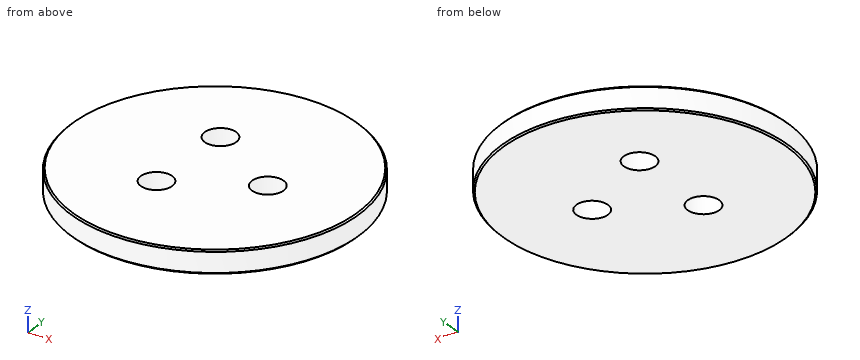
from build123d import *

# Parameters (mm, degrees)
SKETCH1_R           = 100
BOSS_EXTRUDE1_DEPTH = 16
SKETCH2_R           = 11
CUT_EXTRUDE1_DEPTH  = 143.323574997
CIRPATTERN1_COUNT   = 3
CHAMFER1_SIZE       = 1


with BuildPart() as part:
    # Sketch1 → Boss-Extrude1 (new body)
    with BuildSketch(Plane.XY):
        Circle(SKETCH1_R)
    extrude(amount=BOSS_EXTRUDE1_DEPTH)

    # Sketch2 → Cut-Extrude1 (cut, through all)
    with BuildSketch(Plane.XY.offset(16)):
        with Locations((37.5, 0)):
            Circle(SKETCH2_R)
    cut_extrude1 = extrude(amount=-CUT_EXTRUDE1_DEPTH, mode=Mode.SUBTRACT)

    # CirPattern1: Cut-Extrude1 ×3 about axis
    cirpattern1_axis = Axis((0, 0, 0), (0, 0, 1))
    for i in range(1, CIRPATTERN1_COUNT):
        add(cut_extrude1.rotate(cirpattern1_axis, i * 360 / CIRPATTERN1_COUNT), mode=Mode.SUBTRACT)

    # Chamfer1
    chamfer1_edges = [part.edges().sort_by_distance(p)[0] for p in [
        (-100, 0, 0),
        (-100, 0, 16),
    ]]
    chamfer(chamfer1_edges, length=CHAMFER1_SIZE)


solid = part.part
Part model, mm, in its own coordinate system. Give positions to 0.01 mm unless a question says otherwise; leave off trailing zeros. Order: outer loops, then holes, each group sorted by start corner. A loop starts at its lowest first (then second) coordinate and runs counter-clockwise, first axis right, second up. Notation, with made-up numbers: (31.5, -8.5) - (80.5, -8.5) arc R18 ccw to (80.5, 1.5) - close; hole circle Ø3 at (-35.75, 56). An arc over 180 degrees is marked (long way). Use a Markdown table: item, result.
1) Flat gauge pins, fed straight in: P1, Ø3, axis at y = -22.5, z = 2, coming from the +X side; P2, Ø1.5, axis at y = -14.5, z = 6.5, coming from the +X side; P3, Ø1.5, axis at x = 25.5, z = 9, coming from the -Y side; P4, Ø20, axis at x = -18.75, y = -32.48, coming from the +Z side. Where does each tip first touch, or does it go through?
Checked values:
| item | result |
|---|---|
| P1 | x = 97.77 |
| P2 | x = 99.05 |
| P3 | y = -96.89 |
| P4 | through |
2) Saw through at A-A on y = 0. List the corners of the cut face in (x, z), plus the area to 3 significant figures.
Checked values:
| item | result |
|---|---|
| outline | (-100, 1) - (-99, 0) - (26.5, 0) - (26.5, 16) - (-99, 16) - (-100, 15) - close; (48.5, 0) - (99, 0) - (100, 1) - (100, 15) - (99, 16) - (48.5, 16) - close |
| area | 2,850 mm² |
3) Saw through at C-C on x = -18.75. Count the separate pieces of the cut face and the enclosed holes in it, plus the area to 3 significant figures.
Checked values:
| item | result |
|---|---|
| separate pieces | 3 |
| enclosed holes | 0 |
| area | 2,440 mm² |
4) Saw through at B-B on z = 4.25. List the corners of the cut face in (x, y), plus the area to 3 significant figures.
Checked values:
| item | result |
|---|---|
| outline | circle Ø200 at (0, 0); hole circle Ø22 at (-18.75, -32.48); hole circle Ø22 at (-18.75, 32.48); hole circle Ø22 at (37.5, 0) |
| area | 30,300 mm² |
5) Probe L1, parallel to Y at x = -18.75, z = 10.25; L2, parallel to Y at x = 37.5, z = 7.5; L3, parallel to Y at x = -24.5, z = 5.5. List the from-to ranges inside material, lowest first. Write a range as from..to.
Checked values:
| item | result |
|---|---|
| L1 | -98.23..-43.48, -21.48..21.48, 43.48..98.23 |
| L2 | -92.7..-11, 11..92.7 |
| L3 | -96.95..-41.85, -23.1..23.1, 41.85..96.95 |
